Source: CAD feature listing. Evaluate the final solid. Frame: model axes, mm. Face numbers are marked on the shaded views. A direction names the side the tool comes from. Give positions to 0.01 mm unless a question says otherwise; leave off trailing zeros. Order: outer loops, then holes, each group sorted by start corner. A loop starts at its lowest first (then second) coordinate and runs counter-clockwise, first axis right, second up.
from build123d import *

# Parameters (mm, degrees)
SKETCH1_W           = 74
SKETCH1_H           = 50
BOSS_EXTRUDE1_DEPTH = 20
SKETCH2_W           = 40
SKETCH2_H           = 40
CUT_EXTRUDE1_DEPTH  = 0.5
SKETCH3_W           = 10
SKETCH3_H           = 40
BOSS_EXTRUDE2_DEPTH = 3
CHAMFER1_SIZE       = 2
SKETCH4_R           = 3.3
SKETCH4_R_2         = 2.5
CUT_EXTRUDE2_DEPTH  = 51.229473419
SKETCH5_R           = 5.5
CUT_EXTRUDE3_DEPTH  = 15


with BuildPart() as part:
    # Sketch1 → Boss-Extrude1 (new body)
    with BuildSketch(Plane.XY):
        Rectangle(SKETCH1_W, SKETCH1_H)
    extrude(amount=BOSS_EXTRUDE1_DEPTH)

    # Sketch2 → Cut-Extrude1 (cut)
    with BuildSketch(Plane.XY.offset(20)):
        with Locations((12, 0)):
            Rectangle(SKETCH2_W, SKETCH2_H)
    extrude(amount=-CUT_EXTRUDE1_DEPTH, mode=Mode.SUBTRACT)

    # Sketch3 → Boss-Extrude2 (add)
    with BuildSketch(Plane(origin=(0, 0, 0), x_dir=(-1, 0, 0), z_dir=(0, 0, -1))):
        with Locations((-17, 0)):
            Rectangle(SKETCH3_W, SKETCH3_H)
        with Locations((27, 0)):
            Rectangle(SKETCH3_W, SKETCH3_H)
    extrude(amount=BOSS_EXTRUDE2_DEPTH)

    # Chamfer1
    chamfer1_edges = [part.edges().sort_by_distance(p)[0] for p in [
        (22, 20, -1.5),
        (22, -20, -1.5),
        (12, -20, -1.5),
        (12, 20, -1.5),
        (-22, 20, -1.5),
        (-22, -20, -1.5),
        (-32, -20, -1.5),
        (-32, 20, -1.5),
    ]]
    chamfer(chamfer1_edges, length=CHAMFER1_SIZE)

    # Sketch4 → Cut-Extrude2 (cut, through all)
    with BuildSketch(Plane(origin=(0, 0, -3), x_dir=(-1, 0, 0), z_dir=(0, 0, -1))):
        with Locations((-17, 12)):
            Circle(SKETCH4_R)
        with Locations((27, 12)):
            Circle(SKETCH4_R)
        with Locations((-25, 13)):
            Circle(SKETCH4_R_2)
        with Locations((1, 13)):
            Circle(SKETCH4_R_2)
        with Locations((1, -13)):
            Circle(SKETCH4_R_2)
        with Locations((-25, -13)):
            Circle(SKETCH4_R_2)
        with Locations(Location((27, -12, 0), (0, 0, 180))):
            Circle(SKETCH4_R)
        with Locations(Location((-17, -12, 0), (0, 0, 180))):
            Circle(SKETCH4_R)
    extrude(amount=-CUT_EXTRUDE2_DEPTH, mode=Mode.SUBTRACT)

    # Sketch5 → Cut-Extrude3 (cut)
    with BuildSketch(Plane.XY.offset(20)):
        with Locations((-27, 12)):
            Circle(SKETCH5_R)
        with Locations((-27, -12)):
            Circle(SKETCH5_R)
        with Locations((17, 12)):
            Circle(SKETCH5_R)
        with Locations((17, -12)):
            Circle(SKETCH5_R)
    extrude(amount=-CUT_EXTRUDE3_DEPTH, mode=Mode.SUBTRACT)


solid = part.part
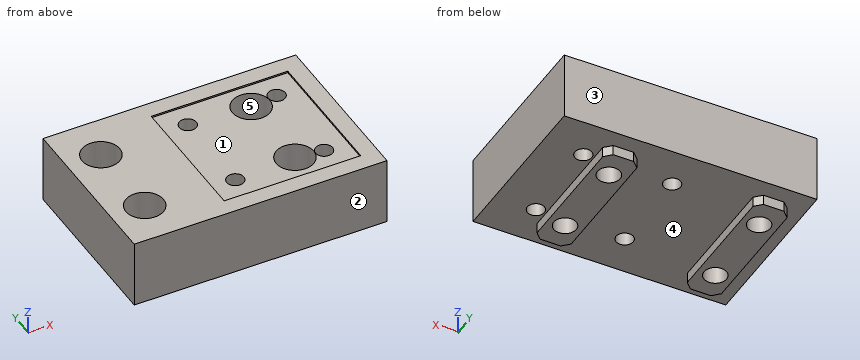
(1) Access query for the marked faces 1 and 2. Directions: +Z, -Z, +X, -X, +Y, -Y. A direction counts if a zero-diameter tool reaches every point of the face in a straight line with its end or side. Return the directions, or none.
(2) Draft query along Y for the marked faces 3, 4 and 5. Return one class per face: +Y half, -Y half, draft (parallel to the pull), parting line (faces both ways), or undercut.
(3) Pin query (flat end, axial travel): pin 1 Ø2.5 at (y, z) = (-3, -2) entering from +X; pin 2 Ø1.5 at (x, y) = (13.5, 0) entering from +Z; pin 3 Ø1.5 at (y, z) = (-5, -1.5) entering from -X. Return the tip coordinate at first contact, or that it passes through.
(4) Line query: line 1 along Y through (x, z) = (17, 0.5); line 2 along Y through (x, z) = (25, 13.75); line 3 along X through (y, z) = (14, 3.25). Output: solid intervals per line, ascending.
(5) Section B-B, the plane z = 7.75. Count the separate pieces of the cut face and the enclosed holes in it, plus the area to 3 significant figures.
(6) Section C-C, the plane y = 3.5. Return loops of the section in (x, z).
(7) Section A-A, the plane x = -27. Return loops of the section in (y, z).
(8) Section D-D, the plane x = -1. Return loops of the section in (y, z).
Checks:
1. face 1: +Z
1. face 2: +Z, -Z, +X, -X, -Y
2. face 3: +Y half
2. face 4: draft
2. face 5: undercut
3. pin 1: stops at x = 22
3. pin 2: stops at z = 19.5
3. pin 3: stops at x = -32
4. line 1: y = -25 to -15.3, -8.7 to 8.7, 15.3 to 25
4. line 2: y = -25 to -15.5, -10.5 to 10.5, 15.5 to 25
4. line 3: x = -37 to -29.62, -24.38 to -3.29, 1.29 to 14.38, 19.62 to 22.71, 27.29 to 37
5. separate pieces: 1
5. enclosed holes: 8
5. area: 3,240 mm2
6. outline: (-37, 0) - (-32, 0) - (-32, -3) - (-22, -3) - (-22, 0) - (12, 0) - (12, -3) - (22, -3) - (22, 0) - (37, 0) - (37, 20) - (32, 20) - (32, 19.5) - (-8, 19.5) - (-8, 20) - (-37, 20) - close
7. outline: (-25, 0) - (-20, 0) - (-20, -3) - (-15.3, -3) - (-15.3, 5) - (-17.5, 5) - (-17.5, 20) - (-25, 20) - close; (-8.7, -3) - (8.7, -3) - (8.7, 5) - (6.5, 5) - (6.5, 20) - (-6.5, 20) - (-6.5, 5) - (-8.7, 5) - close; (15.3, -3) - (20, -3) - (20, 0) - (25, 0) - (25, 20) - (17.5, 20) - (17.5, 5) - (15.3, 5) - close
8. outline: (-25, 0) - (-15.5, 0) - (-15.5, 19.5) - (-20, 19.5) - (-20, 20) - (-25, 20) - close; (-10.5, 0) - (10.5, 0) - (10.5, 19.5) - (-10.5, 19.5) - close; (15.5, 0) - (25, 0) - (25, 20) - (20, 20) - (20, 19.5) - (15.5, 19.5) - close
